```python
from build123d import *

# Parameters (mm, degrees)
EXTRUDE1_DEPTH     = 1000
SKETCH2_R          = 7
CUT_EXTRUDE1_DEPTH = 1004.992031841
LPATTERN1_COUNT    = 3
LPATTERN1_PITCH    = 425


with BuildPart() as part:
    # Sketch1 → Extrude1 (new body)
    with BuildSketch(Plane.XY):
        Polygon((0, 0), (-40, 0), (-40, 80), (0, 80), (0, 76), (-32, 76), (-32, 4), (0, 4), align=None)
    extrude(amount=EXTRUDE1_DEPTH)

    # Sketch2 → Cut-Extrude1 (cut, through all)
    with BuildSketch(Plane(origin=(0, 80, 0), x_dir=(1, 0, 0), z_dir=(0, 1, 0))):
        with Locations(Location((-15, -925, 0), (0, 0, 270))):
            Circle(SKETCH2_R)
    cut_extrude1 = extrude(amount=-CUT_EXTRUDE1_DEPTH, mode=Mode.SUBTRACT)

    # LPattern1: Cut-Extrude1 ×3
    with Locations(*[(0, 0, -i * LPATTERN1_PITCH) for i in range(1, LPATTERN1_COUNT)]):
        add(cut_extrude1, mode=Mode.SUBTRACT)


solid = part.part
```
Can you work these out from the model? Positions are in its coordinate system, mm. A direction names the side the tool comes from. Coordinates: 2 decimals unless noted, no trailing zeros. Write each loop counter-clockwise with the first axis right and the second up, starting at its lowest first coordinate (ties: lowest second). Pieces come first, ordered by that corner, then holes. Notation, with made-up numbers: (68, -19) - (120, -19) arc R8 ccw to (120, -4) - close; hole circle Ø9 at (-34, 41). An arc over 180 degrees is marked (long way). Return JSON: item names as keys, results as strings.
Q1. I'm going to push a flat-ended pin straight in: pin 1 Ø11 at (x, z) = (-15, 500) entering from -Y. Where does the tip first touch, or does it pass through?
Computed values:
{"pin 1": "passes through"}
Q2. If we section it at C-C (y = 36): Please give me the cut outline in (x, z).
Computed values:
{"outline": "(-40, 0) - (-32, 0) - (-32, 1000) - (-40, 1000) - close"}
Q3. Please list where these lines run through material, in increasing order: L1, parallel to Y at x = -23, z = 495.5; L2, parallel to X at y = 2.7, z = 75; L3, parallel to X at y = 71, z = 57.5. Write a range as from..to.
Computed values:
{"L1": "y = 0..4, 76..80", "L2": "x = -40..-22, -8..0", "L3": "x = -40..-32"}
Q4. On a 3-axis mill with a long thin cutter (end or side, diameter ignored), from which of +Z, -Z, +X, -X, +Y, -Y can I reach the whole of each face in a straight line? I mean faces 5 (the flat face through (-19, 76, 493)), 6 (the flat face through (-33, 31, 0)). Say none if no direction works.
Computed values:
{"face 5": "+Z, -Z, +X", "face 6": "-Z, +X, -X, +Y, -Y"}
Q5. If we section it at A-A (x = -15): Count the separate pieces of the cut face and the enclosed holes in it, then the cut area to 3 significant figures.
Computed values:
{"separate pieces": "8", "enclosed holes": "0", "area": "7,660 mm2"}
Q6. Thinking about a two-plate mould opening in Y: for faces 1 (the flat face through (-20, 4, 493)), 2 (the flat face through (-20, 0, 493)), 3 (the flat face through (-20, 80, 493)), 4 (the flat face through (-40, 39, 493)), which applies, +Y half, -Y half, draft (parallel to the pull), parting line (faces both ways), or undercut?
Computed values:
{"face 1": "undercut", "face 2": "-Y half", "face 3": "+Y half", "face 4": "draft"}
Q7. If we section it at B-B (z = 824): Please give me the cut outline in (x, y), then the cut area to 3 significant figures.
Computed values:
{"outline": "(-40, 0) - (0, 0) - (0, 4) - (-32, 4) - (-32, 76) - (0, 76) - (0, 80) - (-40, 80) - close", "area": "896 mm2"}
